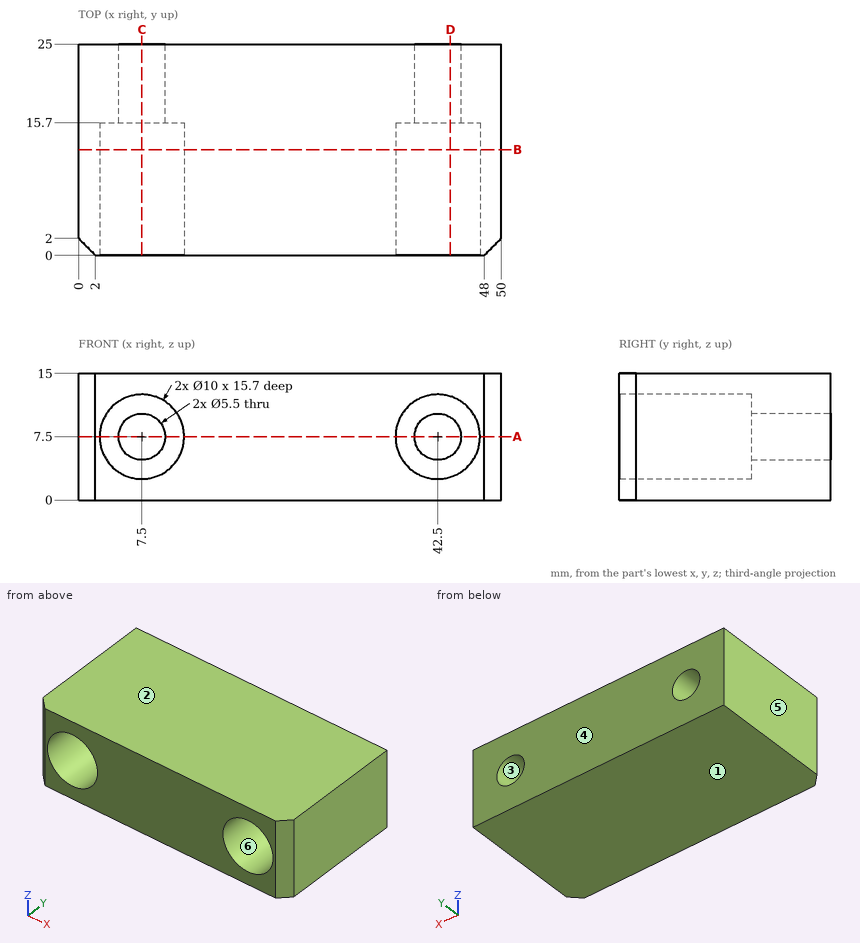
Geometry check sheet. Reference: drawing and pictorial views, mm from the part's lowest x, y, z. A direction names the side the tool comes from. Coordinates: 2 decimals unless noted, no trailing zeros. Write each loop counter-clockwise with the first axis right and the second up, starting at its lowest first coordinate (ties: lowest second). Pieces come first, ordered by that corner, then holes. Notation, with made-up numbers: M -35.75,-12 L 19.25,-12 A27 ccw 19.25,24 Z; hole C 63,-8.75 d2. An arc over 180 degrees is marked long. Write item = value, one per line. Start each with the question number.
1. Tool access check on the marked faces 5 and 6. Record the directions out of +Z, -Z, +X, -X, +Y, -Y that give a thin tool (end or side, any length) a straight path to the whole face; none if there is none.
2. Go/stop test with flat-tipped pins: pin 1 (3 mm diameter, centred on x = 5, z = 6, fed in from -Y); pin 2 (4.5 mm diameter, centred on x = 42.5, z = 7.5, fed in from -Y). Record where each tip stops, or that it passes through.
3. Sectioned sample at A-A (z = 7.5). Record the cut outline in (x, y).
4. Thickness scan on probe 1 along Z at (x, y) = (42.5, 13); probe 2 along X at (y, z) = (3, 5.5); probe 3 along X at (y, z) = (18, 9.25). Record the ranges inside material, lowest first.
5. Mould release check, pull along Z, two halves, no side actions. Record for the marked faces 1, 2, 3 and 4: pulls with the +Z half, pulls with the -Z half, needs draft (parallel to the pull), parting line crosses it, or undercut.
6. Sectioned sample at B-B (y = 12.5). Record the cut outline in (x, z), then the cut area to 3 significant figures.
7. Sectioned sample at C-C (x = 7.5). Record the cut outline in (y, z), then the cut area to 3 significant figures.
8. Sectioned sample at D-D (x = 44). Record the cut outline in (y, z), then the cut area to 3 significant figures.
The answers:
q1.face_5 = +Z, -Z, -X, +Y, -Y
q1.face_6 = -Y
q2.pin_1 = 15.7
q2.pin_2 = through
q3.outline = M 0,2 L 2,0 L 2.5,0 L 2.5,15.7 L 4.75,15.7 L 4.75,25 L 0,25 Z; M 10.25,15.7 L 12.5,15.7 L 12.5,0 L 37.5,0 L 37.5,15.7 L 39.75,15.7 L 39.75,25 L 10.25,25 Z; M 45.25,15.7 L 47.5,15.7 L 47.5,0 L 48,0 L 50,2 L 50,25 L 45.25,25 Z
q4.probe_1 = 0 to 2.5, 12.5 to 15
q4.probe_2 = 0 to 2.92, 12.08 to 37.92, 47.08 to 50
q4.probe_3 = 0 to 5.38, 9.62 to 40.38, 44.62 to 50
q5.face_1 = pulls with the -Z half
q5.face_2 = pulls with the +Z half
q5.face_3 = undercut
q5.face_4 = needs draft
q6.outline = M 0,0 L 50,0 L 50,15 L 0,15 Z; hole C 7.5,7.5 d10; hole C 42.5,7.5 d10
q6.area = 593 mm²
q7.outline = M 0,0 L 25,0 L 25,4.75 L 15.7,4.75 L 15.7,2.5 L 0,2.5 Z; M 0,12.5 L 15.7,12.5 L 15.7,10.25 L 25,10.25 L 25,15 L 0,15 Z
q7.area = 167 mm²
q8.outline = M 0,0 L 25,0 L 25,5.2 L 15.7,5.2 L 15.7,2.73 L 0,2.73 Z; M 0,12.27 L 15.7,12.27 L 15.7,9.8 L 25,9.8 L 25,15 L 0,15 Z
q8.area = 182 mm²
